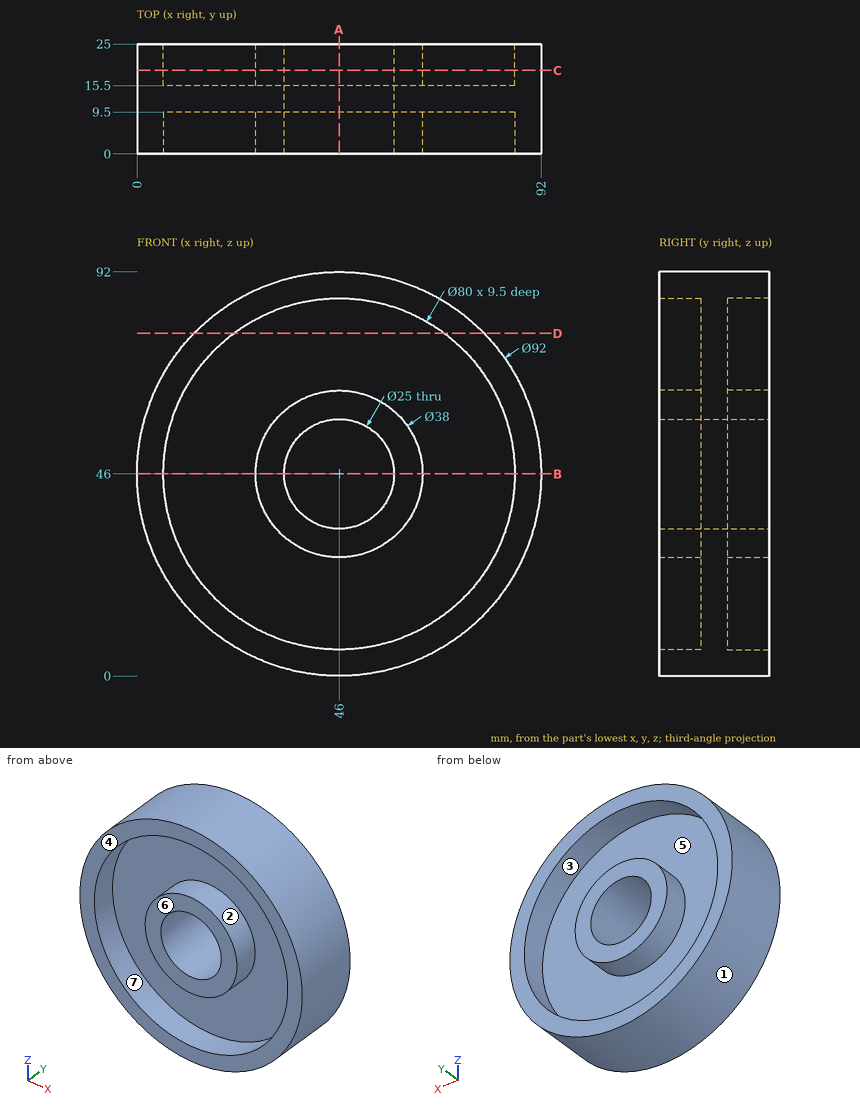
Study the drawing (mm; zero at the part's minimum x, y, z) and answer. A direction names the side the tool comes from. Coordinates: 2 decimals unless noted, no trailing zeros. Loops run counter-clockwise (first coordinate to the right, second up) from the corner with the lowest first, then second, coordinate; pieces in that order, holes last. Notation, with made-up numbers: (-23.5, 46.25) -> (33.5, 46.25) arc R10 cw to (33.5, 53.25) -> close; hole circle Ø11 at (28.25, 83). An arc over 180 degrees is marked (long way). Write each question's results on one line, items separated by ' | '. Start each with the question number.
1) Flat-ended cylindrical pins translate along their axes: P1, Ø5, axis at y = 14, z = 58.5, coming from the -X side; P2, Ø4, axis at x = 69, y = 16, coming from the +Z side; P3, Ø15, axis at x = 46, z = 46, coming from the +Y side; P4, Ø1.5, axis at x = 66.5, z = 20.5, coming from the +Y side. Find the tip coordinate at first contact, or state that the pin passes through.
2) Find section C-C on y = 19. Determine the outline of the cut face in (x, z).
3) Find section D-D on z = 78. Determine the outline of the cut face in (x, y).
4) Consider line 1 along X through (y, z) = (5.75, 46); line 2 along X through (y, z) = (19.25, 47.5); line 3 along Z through (x, y) = (38, 6). Determine where each line is inside the solid, lowest interval first.
5) Find section B-B on z = 46. Determine the outline of the cut face in (x, y), then the cut area to 3 significant figures.
6) The mould has two halves that part along X. Classify the marked faces 1, 2, 3 and 4: pulls with the +X half, pulls with the -X half, needs draft (parallel to the pull), parting line crosses it, or undercut.
7) For the marked faces 5, 6 and 7, determine the directions among +Z, -Z, +X, -X, +Y, -Y from which every point of the face is accessible in a straight line to the end or side of a thin tool.
8) Find section A-A on x = 46. Determine the outline of the cut face in (y, z), then the cut area to 3 significant figures.
Response values:
1) P1: stops at x = 1.1 | P2: stops at z = 86.93 | P3: passes through | P4: stops at y = 15.5
2) outline: circle Ø92 at (46, 46); circle Ø38 at (46, 46); hole circle Ø80 at (46, 46); hole circle Ø25 at (46, 46)
3) outline: (12.95, 0) -> (22, 0) -> (22, 9.5) -> (70, 9.5) -> (70, 0) -> (79.05, 0) -> (79.05, 25) -> (70, 25) -> (70, 15.5) -> (22, 15.5) -> (22, 25) -> (12.95, 25) -> close
4) line 1: x = 0 to 6, 27 to 33.5, 58.5 to 65, 86 to 92 | line 2: x = 0.02 to 6.03, 27.06 to 33.59, 58.41 to 64.94, 85.97 to 91.98 | line 3: z = 0.7 to 6.81, 28.77 to 36.4, 55.6 to 63.23, 85.19 to 91.3
5) outline: (0, 0) -> (6, 0) -> (6, 9.5) -> (27, 9.5) -> (27, 0) -> (33.5, 0) -> (33.5, 25) -> (27, 25) -> (27, 15.5) -> (6, 15.5) -> (6, 25) -> (0, 25) -> close; (58.5, 0) -> (65, 0) -> (65, 9.5) -> (86, 9.5) -> (86, 0) -> (92, 0) -> (92, 25) -> (86, 25) -> (86, 15.5) -> (65, 15.5) -> (65, 25) -> (58.5, 25) -> close | area: 877 mm^2
6) face 1: parting line crosses it | face 2: undercut | face 3: undercut | face 4: needs draft
7) face 5: +Y | face 6: +Z, -Z, +X, -X, -Y | face 7: -Y
8) outline: (0, 0) -> (25, 0) -> (25, 6) -> (15.5, 6) -> (15.5, 27) -> (25, 27) -> (25, 33.5) -> (0, 33.5) -> (0, 27) -> (9.5, 27) -> (9.5, 6) -> (0, 6) -> close; (0, 58.5) -> (25, 58.5) -> (25, 65) -> (15.5, 65) -> (15.5, 86) -> (25, 86) -> (25, 92) -> (0, 92) -> (0, 86) -> (9.5, 86) -> (9.5, 65) -> (0, 65) -> close | area: 877 mm^2
